```python
from build123d import *

# Parameters (mm, degrees)
SKETCH_1_R             = 9
EXTRUDE_1_DEPTH        = 34
SKETCH_2_R             = 8
EXTRUDE_2_DEPTH        = 3
SKETCH_3_R             = 10.5
EXTRUDE_3_DEPTH        = 2
EXTRUDE_START          = 21
SKETCH_4_R             = 8
EXTRUDE_4_DEPTH        = 21
SKETCH_5_W             = 5
SKETCH_5_H             = 32.45039325
CUT_EXTRUDE_1_DEPTH    = 3
HOLE_WIZARD_M8_1_D     = 6.8
HOLE_WIZARD_M8_1_DEPTH = 19.75
HOLE_WIZARD_M8_1_TIP   = 2.042926105
CHAMFER_1_SIZE         = 0.2


with BuildPart() as part:
    # 草图1 → 凸台-拉伸1 (new body)
    with BuildSketch(Plane.XY):
        Circle(SKETCH_1_R)
    extrude(amount=EXTRUDE_1_DEPTH)

    # 草图2 → 凸台-拉伸2 (add)
    with BuildSketch(Plane.XY.offset(34)):
        Circle(SKETCH_2_R)
    extrude(amount=EXTRUDE_2_DEPTH)

    # 草图3 → 凸台-拉伸3 (add)
    with BuildSketch(Plane(origin=(0, 0, 0), x_dir=(-1, 0, 0), z_dir=(0, 0, -1))):
        Circle(SKETCH_3_R)
    extrude(amount=EXTRUDE_3_DEPTH)

    # 草图4 → 凸台-拉伸4 (add)
    with BuildSketch(Plane(origin=(0, 0, -2), x_dir=(-1, 0, 0), z_dir=(0, 0, -1)).offset(EXTRUDE_START)):
        with Locations(Location((0, 0, 0), (0, 0, 180))):
            Circle(SKETCH_4_R)
    extrude(amount=-EXTRUDE_4_DEPTH)

    # 草图5 → 切除-拉伸1 (cut)
    with BuildSketch(Plane.XY.offset(37)):
        with Locations((0, 1.931578492)):
            Rectangle(SKETCH_5_W, SKETCH_5_H)
    extrude(amount=-CUT_EXTRUDE_1_DEPTH, mode=Mode.SUBTRACT)

    # M8 螺纹孔1
    with Locations(Plane.XY.offset(37)):
        with Locations((0, 0)):
            Hole(HOLE_WIZARD_M8_1_D / 2, depth=HOLE_WIZARD_M8_1_DEPTH)
            with Locations((0, 0, -(HOLE_WIZARD_M8_1_DEPTH + HOLE_WIZARD_M8_1_TIP / 2))):  # 118° drill point
                Cone(0, HOLE_WIZARD_M8_1_D / 2, HOLE_WIZARD_M8_1_TIP, mode=Mode.SUBTRACT)

    # 倒角1
    chamfer_1_edges = [part.edges().sort_by_distance(p)[0] for p in [
        (10.5, 0, -2),
        (-8, 0, -23),
        (-9, 0, 34),
        (-8, 0, 37),
        (8, 0, 37),
        (10.5, 0, 0),
    ]]
    chamfer(chamfer_1_edges, length=CHAMFER_1_SIZE)


solid = part.part
```
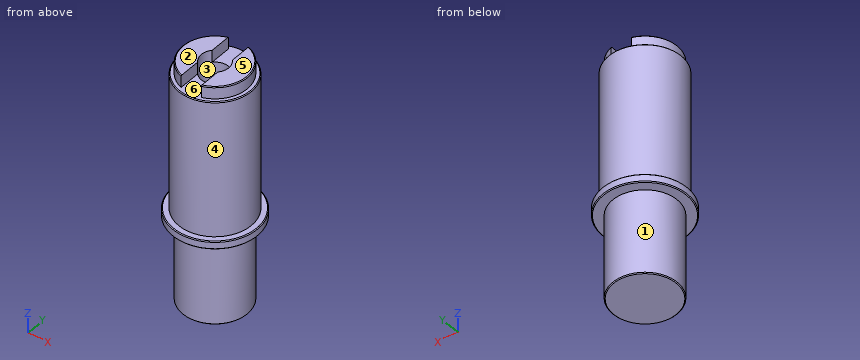
Source: CAD feature listing. Evaluate the final solid. Frame: model axes, mm. Face numbers are marked on the shaded views. A direction names the side the tool comes from. Round coordinates to 2 decimals unless told otherwise and drop trailing zeros. Loops run counter-clockwise (first coordinate to the right, second up) from the corner with the lowest first, then second, coordinate; pieces in that order, holes last. Notation, with made-up numbers: M 88,-24 L 136,-24 A21 ccw 136,14 Z; hole C 46,-13.75 d9. An arc over 180 degrees is marked long. Use a Markdown table: item, result. Add a question column.
1. Section query C-C on z = -15. Return the cut outline in (x, y).
2. Contact query for flat-ended pins moving along their axis: P1, Ø6, axis at x = -2, y = -3, coming from the +Z side; P2, Ø4, axis at x = 5, z = -0.5, coming from the -Y side; P3, Ø2.5, axis at y = -5, z = 36, coming from the -X side; P4, Ø10, axis at x = 7.5, z = 12.5, coming from the +Y side. Output: stop coordinate, or through.
3. Line query: line 1 (X direction, y = 0, z = 26.5); line 2 (Y direction, x = -0.25, z = -9). Output: solid intervals per line, ascending.
4. Section query A-A on z = 32. Return the cut outline in (x, y), then the cut area to 3 significant figures.
5. Section query B-B on z = 13. Return the cut outline in (x, y), then the cut area to 3 significant figures.
6. Reachability of the marked faces 1, 2 and 3 from +Z, -Z, +X, -X, +Y, -Y: full face, straight path, thin tool, end or side. Return the list, or none.
7. Mould query, pull axis X, two halves, no side actions, for the marked faces 4, 5 and 6. Classes: pulls with the +X half, pulls with the -X half, needs draft (parallel to the pull), parting line crosses it, or undercut.
Reported:
| question | item | result |
|---|---|---|
| 1 | outline | C 0,0 d16 |
| 2 | P1 | stops at z = 37 |
| 2 | P2 | stops at y = -10.06 |
| 2 | P3 | stops at x = -7.07 |
| 2 | P4 | stops at y = 8.65 |
| 3 | line 1 | x = -9 to -3.4, 3.4 to 9 |
| 3 | line 2 | y = -8 to 8 |
| 4 | outline | C 0,0 d18; hole C 0,0 d6.8 |
| 4 | area | 218 mm² |
| 5 | outline | C 0,0 d18 |
| 5 | area | 254 mm² |
| 6 | face 1 | -Z |
| 6 | face 2 | +Z, +X, -X, +Y, -Y |
| 6 | face 3 | +Z |
| 7 | face 4 | parting line crosses it |
| 7 | face 5 | needs draft |
| 7 | face 6 | undercut |
